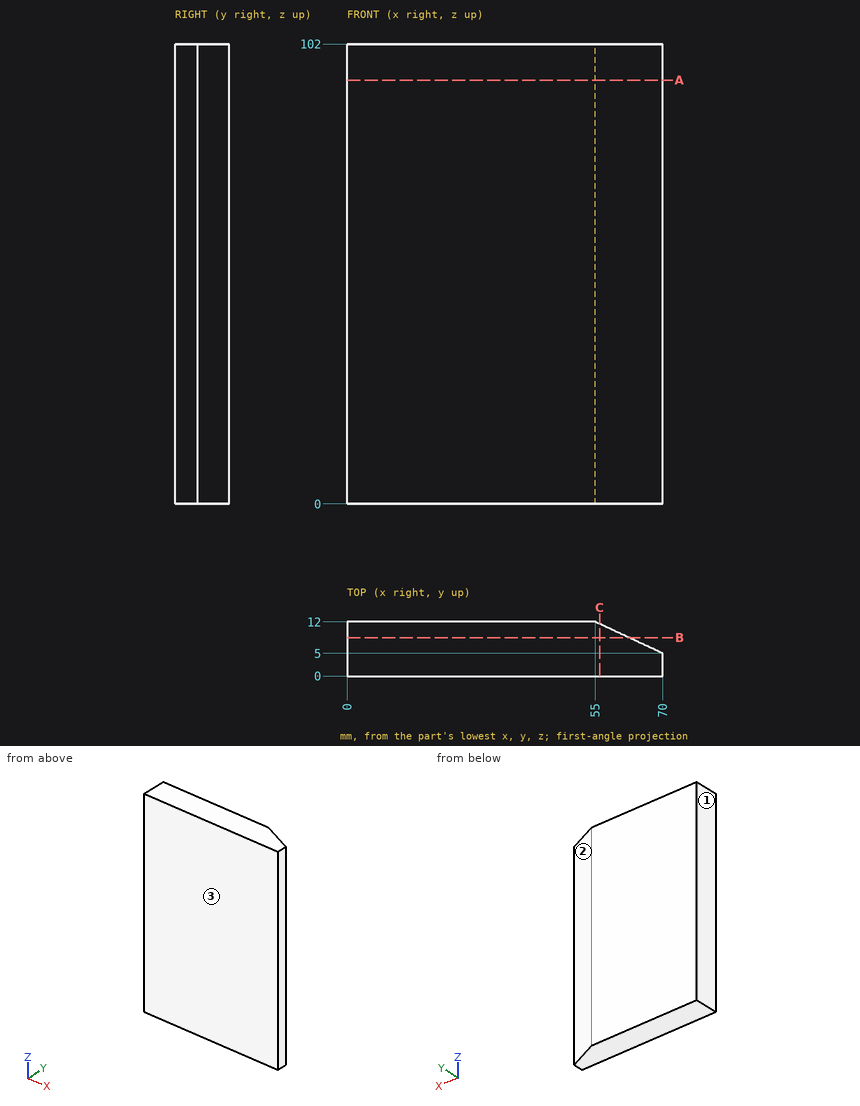
The figure shows three views and two pictorial views of one solid part (mm, origin at its lowest corner). Answer the questions. Round coordinates to 2 decimals unless told otherwise and drop trailing zeros. Order: outer loops, then holes, each group sorted by start corner. A loop starts at its lowest first (then second) coordinate and runs counter-clockwise, first axis right, second up.
Q1. Given pin 1 Ø1 at (y, z) = (10, 35.5) entering from -X, flat-ended and moving along its own axis, determine where the tip first touches the part or whether it passes through.
Solution:
pin 1: stops at x = 0
Q2. A cutting plane is placed at B-B, the plane y = 8.5. Determine the outline of the cut face in (x, z).
Solution:
outline: (0, 0) - (62.5, 0) - (62.5, 102) - (0, 102) - close
Q3. Find the intervals of material crossed by line 1 along X through (y, z) = (8.5, 45); line 2 along X through (y, z) = (5.75, 93); line 3 along Y through (x, z) = (59.5, 12.5), in increasing order.
Solution:
line 1: x = 0 to 62.5
line 2: x = 0 to 68.39
line 3: y = 0 to 9.9
Q4. A cutting plane is placed at C-C, the plane x = 56. Determine the outline of the cut face in (y, z).
Solution:
outline: (0, 0) - (11.53, 0) - (11.53, 102) - (0, 102) - close
Q5. The mould has two halves that part along X. Classify the marked faces 1, 2 and 3: pulls with the +X half, pulls with the -X half, needs draft (parallel to the pull), parting line crosses it, or undercut.
Solution:
face 1: pulls with the -X half
face 2: pulls with the +X half
face 3: needs draft
Q6. A cutting plane is placed at A-A, the plane z = 94. Determine the outline of the cut face in (x, y), then the cut area to 4 significant figures.
Solution:
outline: (0, 0) - (70, 0) - (70, 5) - (55, 12) - (0, 12) - close
area: 787.5 mm2
